```python
from build123d import *

# Parameters (mm, degrees)
GB_T6728_2002_70_70_5_1_DEPTH = 476
CUT_EXTRUDE_1_DEPTH           = 483.390920313
CUT_EXTRUDE_1_DEPTH_BACK      = 483.390920313


with BuildPart() as part:
    # Sketch1 → 结构用冷弯空心方钢(gb t6728-2002) 70×70×5(1) (new body)
    with BuildSketch(Plane(origin=(0, 0, 0), x_dir=(-1, 0, 0), z_dir=(0, 1, 0))):
        with BuildLine():
            Line((-25, -35), (25, -35))
            ThreePointArc((25, -35), (32.071067812, -32.071067812), (35, -25))
            Line((35, -25), (35, 25))
            ThreePointArc((35, 25), (32.071067812, 32.071067812), (25, 35))
            Line((25, 35), (-25, 35))
            ThreePointArc((-25, 35), (-32.071067812, 32.071067812), (-35, 25))
            Line((-35, 25), (-35, -25))
            ThreePointArc((-35, -25), (-32.071067812, -32.071067812), (-25, -35))
        make_face()
        with BuildLine():
            Line((-25, -30), (25, -30))
            ThreePointArc((25, -30), (28.535533906, -28.535533906), (30, -25))
            Line((30, -25), (30, 25))
            ThreePointArc((30, 25), (28.535533906, 28.535533906), (25, 30))
            Line((25, 30), (-25, 30))
            ThreePointArc((-25, 30), (-28.535533906, 28.535533906), (-30, 25))
            Line((-30, 25), (-30, -25))
            ThreePointArc((-30, -25), (-28.535533906, -28.535533906), (-25, -30))
        make_face(mode=Mode.SUBTRACT)
    extrude(amount=GB_T6728_2002_70_70_5_1_DEPTH)

    # 草图2 → 切除-拉伸1 (cut, two sides: drawn at the far end of the back side and taken through both)
    with BuildSketch(Plane.XY.offset(35).offset(-CUT_EXTRUDE_1_DEPTH_BACK)):
        Polygon((35, 476), (-35, 359.333333333), (-35, 476), align=None)
        Polygon((-35, 42), (35, 0), (-35, 0), align=None)
    extrude(amount=CUT_EXTRUDE_1_DEPTH + CUT_EXTRUDE_1_DEPTH_BACK, mode=Mode.SUBTRACT)


solid = part.part
```
Verification items for the finished model (mm, model axes). A direction names the side the tool comes from. Coordinates: 2 decimals unless noted, no trailing zeros. Loops run counter-clockwise (first coordinate to the right, second up) from the corner with the lowest first, then second, coordinate; pieces in that order, holes last. Notation, with made-up numbers: (83, -36.5) - (114, -36.5) arc R24 cw to (114, 0.5) - close; hole circle Ø1 at (-3.75, 44). An arc over 180 degrees is marked (long way). Answer as a JSON object with one key per item and string values.
(1) Access from +Z, -Z, +X, -X, +Y, -Y to the whole of each face (thin tool, end or side, straight path). Record for faces 1 (the flat face through (0, 229, 30)), 2 (the cylindrical face through (-31.99, 203.62, -32.15)).
Response:
{"face 1": "+Y, -Y", "face 2": "-Z, -X, +Y, -Y"}
(2) Mould release check, pull along Z, two halves, no side actions. Record for faces 3 (the flat face through (0, 229, -30)), 4 (the cylindrical face through (-32.15, 203.62, 31.99)), 5 (the flat face through (0, 21, 31)), 6 (the flat face through (0, 229, -35)): pulls with the +Z half, pulls with the -Z half, needs draft (parallel to the pull), parting line crosses it, or undercut.
Response:
{"face 3": "undercut", "face 4": "pulls with the +Z half", "face 5": "needs draft", "face 6": "pulls with the -Z half"}
(3) Cross-section at A-A, the plane x = -14.5. Record the boundary of the cut face in (y, z), then the cut area to 3 significant figures.
Response:
{"outline": "(29.7, -35) - (393.5, -35) - (393.5, -30) - (29.7, -30) - close; (29.7, 30) - (393.5, 30) - (393.5, 35) - (29.7, 35) - close", "area": "3,640 mm²"}
(4) Go/stop test with a flat-tipped pin: pin 1 Ø3 at (y, z) = (408.5, 11) entering from -X. Record where the tip stops, or that it passes through.
Response:
{"pin 1": "stops at x = 30"}
(5) Scan lines: line 1 along Z through (x, y) = (-6, 52); line 2 along X through (y, z) = (420.5, 13.5). Record each from-to range of solid material in increasing order.
Response:
{"line 1": "z = -35 to -30, 30 to 35", "line 2": "x = 30 to 35"}
(6) Cross-section at B-B, the plane y = 348. Record the boundary of the cut face in (x, z).
Response:
{"outline": "(-35, -25) arc R10 ccw to (-25, -35) - (25, -35) arc R10 ccw to (35, -25) - (35, 25) arc R10 ccw to (25, 35) - (-25, 35) arc R10 ccw to (-35, 25) - close; hole (-30, -25) arc R5 ccw to (-25, -30) - (25, -30) arc R5 ccw to (30, -25) - (30, 25) arc R5 ccw to (25, 30) - (-25, 30) arc R5 ccw to (-30, 25) - close"}
(7) Cross-section at C-C, the plane z = -4. Record the boundary of the cut face in (x, y).
Response:
{"outline": "(-35, 42) - (-30, 39) - (-30, 367.67) - (-35, 359.33) - close; (30, 3) - (35, 0) - (35, 476) - (30, 467.67) - close"}
